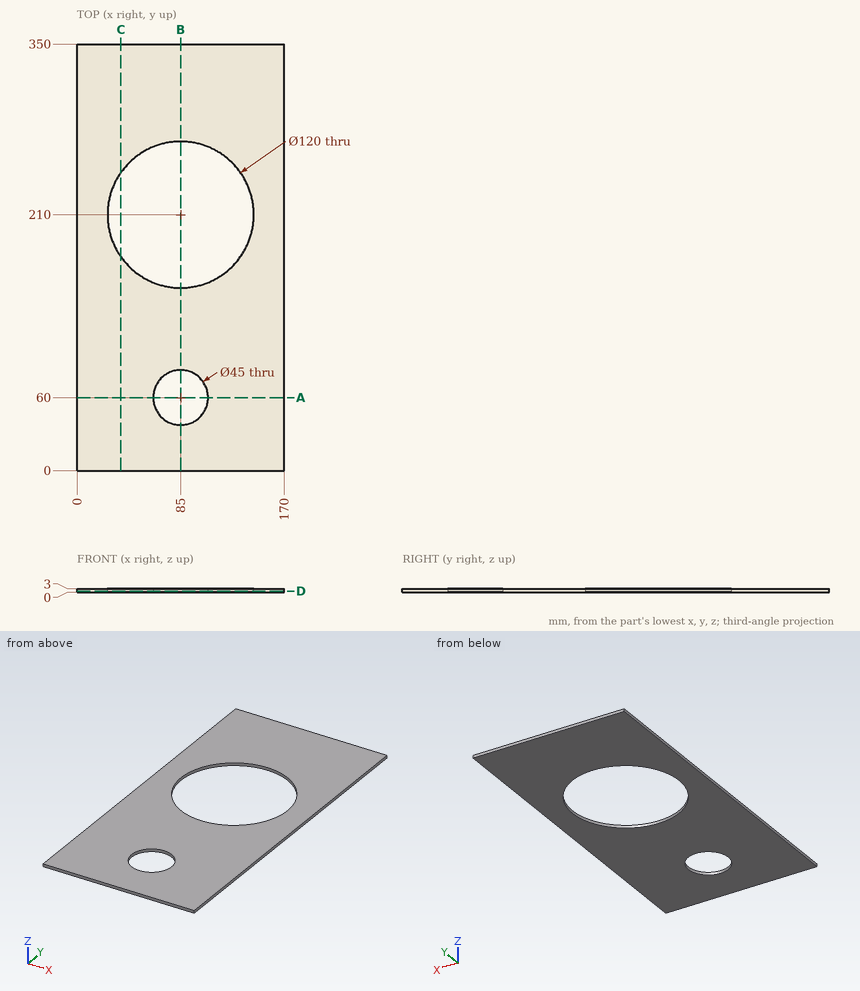
Part print with two shaded views. Sizes in mm from the minimum x, y, z corner. Coordinates: 2 decimals unless noted, no trailing zeros. Write each loop counter-clockwise with the first axis right and the second up, starting at its lowest first coordinate (ties: lowest second). Pieces come first, ordered by that corner, then holes. Notation, with made-up numbers: M 46.5,77.25 L 56.5,77.25 A25 ccw 56.5,92.25 Z; hole C 68,-9 d4. An arc over 180 degrees is marked long. Return JSON: item names as keys, results as strings.
Item 1: Slice it at B-B, the plane x = 85. Write the cut outline in (y, z).
Findings below:
{"outline": "M 0,0 L 37.5,0 L 37.5,3 L 0,3 Z; M 82.5,0 L 150,0 L 150,3 L 82.5,3 Z; M 270,0 L 350,0 L 350,3 L 270,3 Z"}
Item 2: Drop a flat-ended pin along its axis: pin 1 Ø1 at (x, y) = (148, 258.5) entering from -Z. Give the stop position or say it passes through.
Findings below:
{"pin 1": "stops at z = 0"}
Item 3: Probe line 1 (Y direction, x = 85, z = 1.9); line 2 (Y direction, x = 98, z = 2.5); line 3 (X direction, y = 74.5, z = 2.1). List the from-to ranges inside material, lowest first. Write a range as from..to.
Findings below:
{"line 1": "y = 0..37.5, 82.5..150, 270..350", "line 2": "y = 0..41.64, 78.36..151.43, 268.57..350", "line 3": "x = 0..67.8, 102.2..170"}
Item 4: Slice it at A-A, the plane y = 60. Write the cut outline in (x, z), and give its area (3 significant figures).
Findings below:
{"outline": "M 0,0 L 62.5,0 L 62.5,3 L 0,3 Z; M 107.5,0 L 170,0 L 170,3 L 107.5,3 Z", "area": "375 mm2"}
Item 5: Slice it at C-C, the plane x = 36. Write the cut outline in (y, z).
Findings below:
{"outline": "M 0,0 L 175.37,0 L 175.37,3 L 0,3 Z; M 244.63,0 L 350,0 L 350,3 L 244.63,3 Z"}
Item 6: Slice it at D-D, the plane z = 0.95. Write the cut outline in (x, y), and give its area (3 significant figures).
Findings below:
{"outline": "M 0,0 L 170,0 L 170,350 L 0,350 Z; hole C 85,210 d120; hole C 85,60 d45", "area": "46,600 mm2"}
